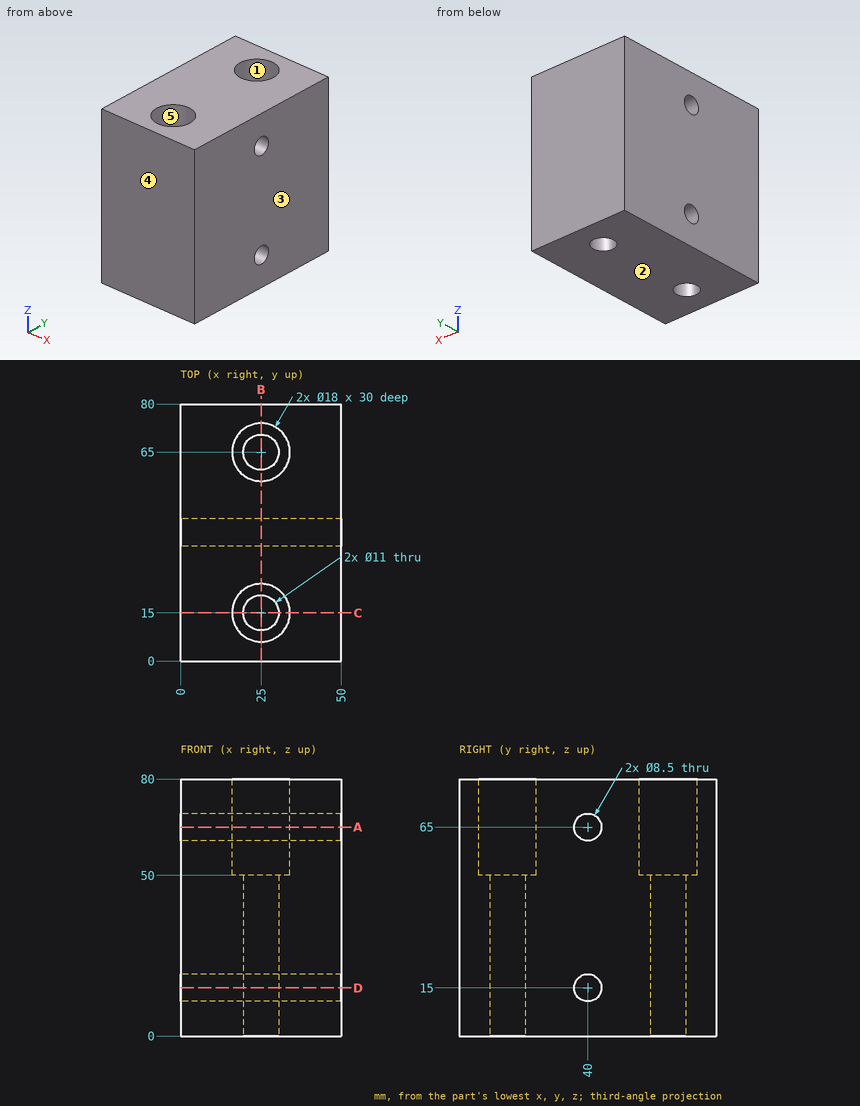
Job drawing, mm, ordinate dimensions from the low corner. One solid piece. A direction names the side the tool comes from. Give positions to 0.01 mm unless a question says otherwise; leave off trailing zeros. Loops run counter-clockwise (first coordinate to the right, second up) from the corner with the lowest first, then second, coordinate; pieces in that order, holes last. Notation, with made-up numbers: (-31.75, 54) -> (7.25, 54) arc R26 ccw to (7.25, 73) -> close; hole circle Ø10 at (-24, 3.25). An arc over 180 degrees is marked (long way). Write each question's results on one line, items separated by ' | '. Start each with the question number.
Q1. Band-saw the part on C-C on y = 15. List the corners of the cut face in (x, z).
Q2. Wall check: L1, parallel to Y at x = 25, z = 70; L2, parallel to Y at x = 25, z = 34; L3, parallel to Z at x = 24, y = 38.5. Give the ranges that are in metal, low to high.
Q3. Band-saw the part on A-A on z = 65. List the corners of the cut face in (x, y), plus the area to 3 significant figures.
Q4. Band-saw the part on D-D on z = 15. List the corners of the cut face in (x, y).
Q5. Band-saw the part on B-B on x = 25. List the corners of the cut face in (y, z).
Q6. Pull direction X, two halves, no side cores. Call the marked faces 3, 4 and 5: +X half, -X half, draft (parallel to the pull), parting line (faces both ways), or undercut.
Q7. Which spindle directions (+Z, -Z, +X, -X, +Y, -Y) get a long thin tool onto all of the face, cutting with end or side? Do the marked faces 1 and 2. Say none if no direction does.
Q8. Pin check, flat tips, straight feed: P1, Ø6, axis at x = 24, y = 23, coming from the -Z side; P2, Ø14.5, axis at x = 25, y = 15, coming from the +Z side; P3, Ø6.5, axis at x = 25, y = 15, coming from the -Z side. Stop position of each tip, or through.
Results are:
1) outline: (0, 0) -> (19.5, 0) -> (19.5, 50) -> (16, 50) -> (16, 80) -> (0, 80) -> close; (30.5, 0) -> (50, 0) -> (50, 80) -> (34, 80) -> (34, 50) -> (30.5, 50) -> close
2) L1: y = 0 to 6, 24 to 56, 74 to 80 | L2: y = 0 to 9.5, 20.5 to 59.5, 70.5 to 80 | L3: z = 0 to 11.02, 18.98 to 61.02, 68.98 to 80
3) outline: (0, 0) -> (50, 0) -> (50, 35.75) -> (0, 35.75) -> close; (0, 44.25) -> (50, 44.25) -> (50, 80) -> (0, 80) -> close; hole circle Ø18 at (25, 15); hole circle Ø18 at (25, 65) | area: 3,070 mm²
4) outline: (0, 0) -> (50, 0) -> (50, 35.75) -> (0, 35.75) -> close; (0, 44.25) -> (50, 44.25) -> (50, 80) -> (0, 80) -> close; hole circle Ø11 at (25, 15); hole circle Ø11 at (25, 65)
5) outline: (0, 0) -> (9.5, 0) -> (9.5, 50) -> (6, 50) -> (6, 80) -> (0, 80) -> close; (20.5, 0) -> (59.5, 0) -> (59.5, 50) -> (56, 50) -> (56, 80) -> (24, 80) -> (24, 50) -> (20.5, 50) -> close; (70.5, 0) -> (80, 0) -> (80, 80) -> (74, 80) -> (74, 50) -> (70.5, 50) -> close; hole circle Ø8.5 at (40, 15); hole circle Ø8.5 at (40, 65)
6) face 3: +X half | face 4: draft | face 5: undercut
7) face 1: +Z | face 2: -Z, +X, -X, +Y, -Y
8) P1: stops at z = 0 | P2: stops at z = 50 | P3: passes through
